Input: dimensioned drawing with shaded views. Units: mm. Origin: part minimum x, y, z. Coordinates: 2 decimals unless noted, no trailing zeros. Order: outer loops, then holes, each group sorted by start corner. A loop starts at its lowest first (then second) coordinate and runs counter-clockwise, first axis right, second up. Notation, with made-up numbers: (23, -10.75) -> (59, -10.75) arc R33 cw to (59, 21.25) -> close; hole circle Ø2 at (-18, -34). An arc over 180 degrees is marked (long way). Put each result on its own line as item: value.
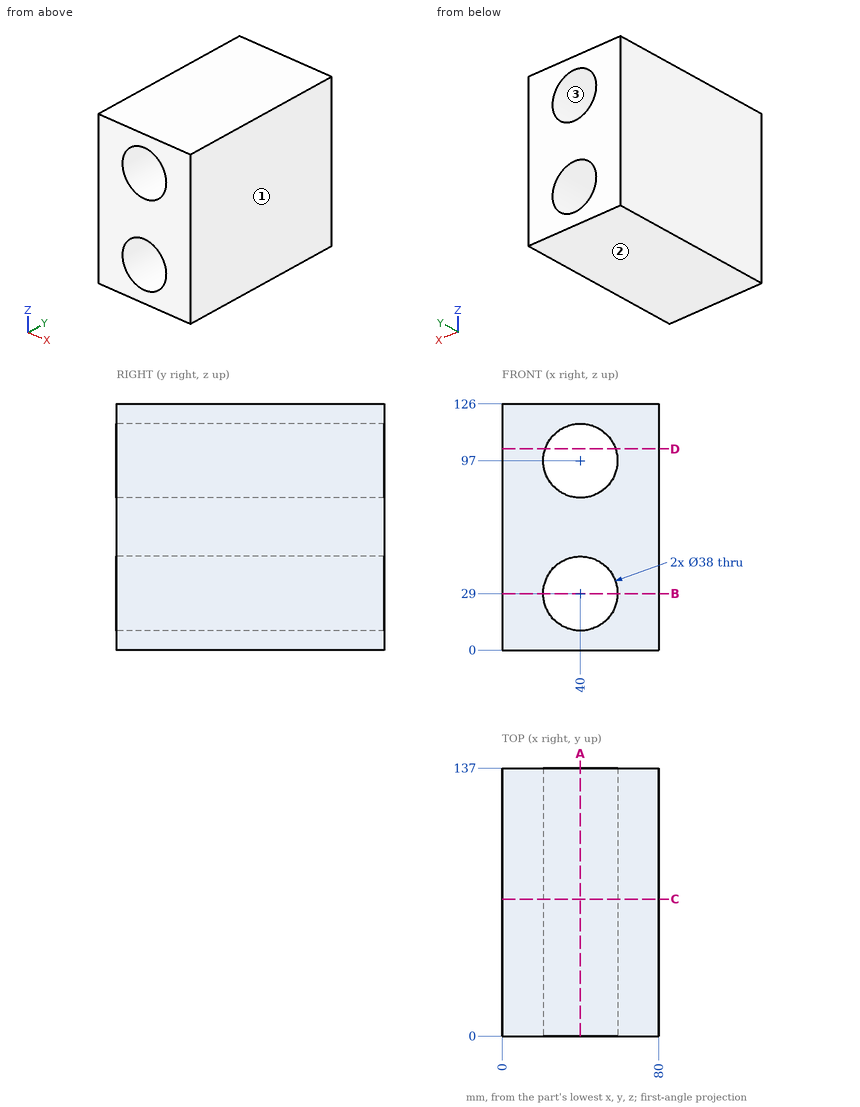
1. Cut plane C-C on y = 70. Output: boundary loops of the cut face in (x, z), plus the area to 3 significant figures.
Numbers:
outline: (0, 0) -> (80, 0) -> (80, 126) -> (0, 126) -> close; hole circle Ø38 at (40, 29); hole circle Ø38 at (40, 97)
area: 7,810 mm2
2. Ray query, line 1 along X through (y, z) = (100, 97); line 2 along Z through (x, y) = (29, 81); line 3 along Z through (x, y) = (30.5, 114). Return the intervals inside material, ascending.
Numbers:
line 1: x = 0 to 21, 59 to 80
line 2: z = 0 to 13.51, 44.49 to 81.51, 112.49 to 126
line 3: z = 0 to 12.55, 45.45 to 80.55, 113.45 to 126
3. Cut plane B-B on z = 29. Output: boundary loops of the cut face in (x, y), plus the area to 3 significant figures.
Numbers:
outline: (0, 0) -> (21, 0) -> (21, 137) -> (0, 137) -> close; (59, 0) -> (80, 0) -> (80, 137) -> (59, 137) -> close
area: 5,750 mm2
4. Cut plane A-A on x = 40. Output: boundary loops of the cut face in (y, z).
Numbers:
outline: (0, 0) -> (137, 0) -> (137, 10) -> (0, 10) -> close; (0, 48) -> (137, 48) -> (137, 78) -> (0, 78) -> close; (0, 116) -> (137, 116) -> (137, 126) -> (0, 126) -> close
5. Cut plane D-D on z = 103. Output: boundary loops of the cut face in (x, y).
Numbers:
outline: (0, 0) -> (21.97, 0) -> (21.97, 137) -> (0, 137) -> close; (58.03, 0) -> (80, 0) -> (80, 137) -> (58.03, 137) -> close
6. First-contact query: pin 1 (2 mm diameter, centred on x = 22.5, z = 33, fed in from +Y). Flat tip, straight axial feed; report the tip coordinate or a pass-through.
Numbers:
pin 1: passes through
7. Pull-direction query (X, two-part tool) for the marked faces 1, 2 and 3; classes: pulls with the +X half, pulls with the -X half, needs draft (parallel to the pull), parting line crosses it, or undercut.
Numbers:
face 1: pulls with the +X half
face 2: needs draft
face 3: undercut
